Can you work these out from the model? Positions are in its coordinate system, mm. Face numbers are marked on the shaded views. A direction names the side the tool comes from. Give positions to 0.01 mm unless a question says otherwise; leave off trailing zeros. Loops run counter-clockwise (first coordinate to the right, second up) from the corner with the lowest first, then second, coordinate; pieces in that order, holes last.
from build123d import *

# Parameters (mm, degrees)
SKETCH_1_W                   = 50
SKETCH_1_H                   = 50
EXTRUDE_1_DEPTH              = 4
SKETCH_2_R                   = 13
CUT_EXTRUDE_1_DEPTH          = 5
HOLE_WIZARD_M5_1_D           = 5.8
HOLE_WIZARD_M5_1_CBORE_D     = 10
HOLE_WIZARD_M5_1_CBORE_DEPTH = 5.4
CHAMFER_1_SIZE               = 2


with BuildPart() as part:
    # 草图1 → 凸台-拉伸1 (new, symmetric)
    with BuildSketch(Plane.XY):
        Rectangle(SKETCH_1_W, SKETCH_1_H)
    extrude(amount=EXTRUDE_1_DEPTH, both=True)

    # 草图2 → 切除-拉伸1 (cut)
    with BuildSketch(Plane.XY.offset(4)):
        Circle(SKETCH_2_R)
    extrude(amount=-CUT_EXTRUDE_1_DEPTH, mode=Mode.SUBTRACT)

    # M5 六角凹头螺钉的柱形沉头孔1 (through all)
    with Locations(Plane(origin=(0, 0, -4), x_dir=(1, 0, 0), z_dir=(0, 0, -1))):
        with Locations((-19, 0), (0, -19), (19, 0), (0, 19)):
            CounterBoreHole(HOLE_WIZARD_M5_1_D / 2, HOLE_WIZARD_M5_1_CBORE_D / 2, HOLE_WIZARD_M5_1_CBORE_DEPTH)

    # 倒角1
    chamfer_1_edges = [part.edges().sort_by_distance(p)[0] for p in [
        (25, -25, 0),
        (-25, -25, 0),
        (-25, 25, 0),
        (25, 25, 0),
    ]]
    chamfer(chamfer_1_edges, length=CHAMFER_1_SIZE)


solid = part.part
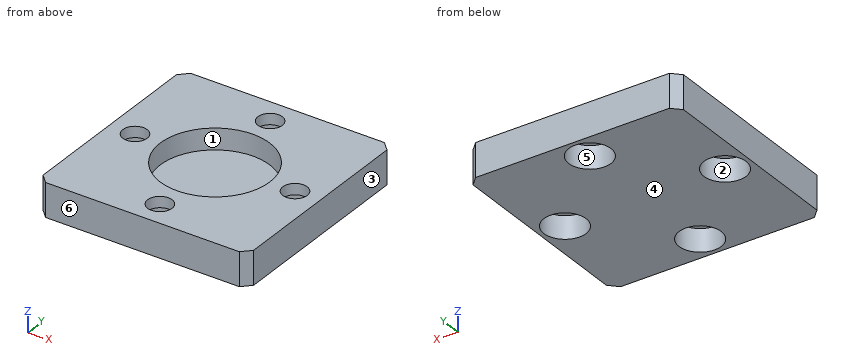
(1) Suppose I cut it at A-A on y = 19. List the corners of the cut face in (x, z) for me, plus the area to 3 significant figures.
Returned:
outline: (-25, -4) - (-5, -4) - (-5, 1.4) - (-2.9, 1.4) - (-2.9, 4) - (-25, 4) - close; (2.9, 1.4) - (5, 1.4) - (5, -4) - (25, -4) - (25, 4) - (2.9, 4) - close
area: 331 mm2
(2) Will these pins go through, and if not, where does the flat tip stop? P1, Ø8, axis at x = -4.5, y = 4, coming from the +Z side; P2, Ø7.5, axis at x = 19, y = 0, coming from the -Z side.
Returned:
P1: stops at z = -1
P2: stops at z = 1.4
(3) Thinking about a two-plate mould opening in Y: for the marked faces 4, 5 and 6, which applies, pulls with the +Y half, pulls with the -Y half, needs draft (parallel to the pull), parting line crosses it, or undercut?
Returned:
face 4: needs draft
face 5: undercut
face 6: pulls with the -Y half
(4) Which directions (+Z, -Z, +X, -X, +Y, -Y) give clear straight access to the entire face, cutting with the end or side of a thin tool? Please do the marked faces 1, 2 and 3.
Returned:
face 1: +Z
face 2: -Z
face 3: +Z, -Z, +X, +Y, -Y
(5) Please list where these lines run through material, in increasing order: probe 1 along Y at (x, z) = (0, 3.1); probe 2 along X at (y, z) = (19, 2.45); probe 3 along X at (y, z) = (-22, -0.25).
Returned:
probe 1: y = -25 to -21.9, -16.1 to -13, 13 to 16.1, 21.9 to 25
probe 2: x = -25 to -2.9, 2.9 to 25
probe 3: x = -25 to -4, 4 to 25
(6) Suppose I cut it at D-D on x = 0. List the corners of the cut face in (y, z) for me.
Returned:
outline: (-25, -4) - (-24, -4) - (-24, 1.4) - (-21.9, 1.4) - (-21.9, 4) - (-25, 4) - close; (-16.1, 1.4) - (-14, 1.4) - (-14, -4) - (14, -4) - (14, 1.4) - (16.1, 1.4) - (16.1, 4) - (13, 4) - (13, -1) - (-13, -1) - (-13, 4) - (-16.1, 4) - close; (21.9, 1.4) - (24, 1.4) - (24, -4) - (25, -4) - (25, 4) - (21.9, 4) - close
(7) Suppose I cut it at B-B on z = -3. List the corners of the cut face in (x, y) for me.
Returned:
outline: (-25, -23) - (-23, -25) - (23, -25) - (25, -23) - (25, 23) - (23, 25) - (-23, 25) - (-25, 23) - close; hole circle Ø10 at (-19, 0); hole circle Ø10 at (0, -19); hole circle Ø10 at (0, 19); hole circle Ø10 at (19, 0)
